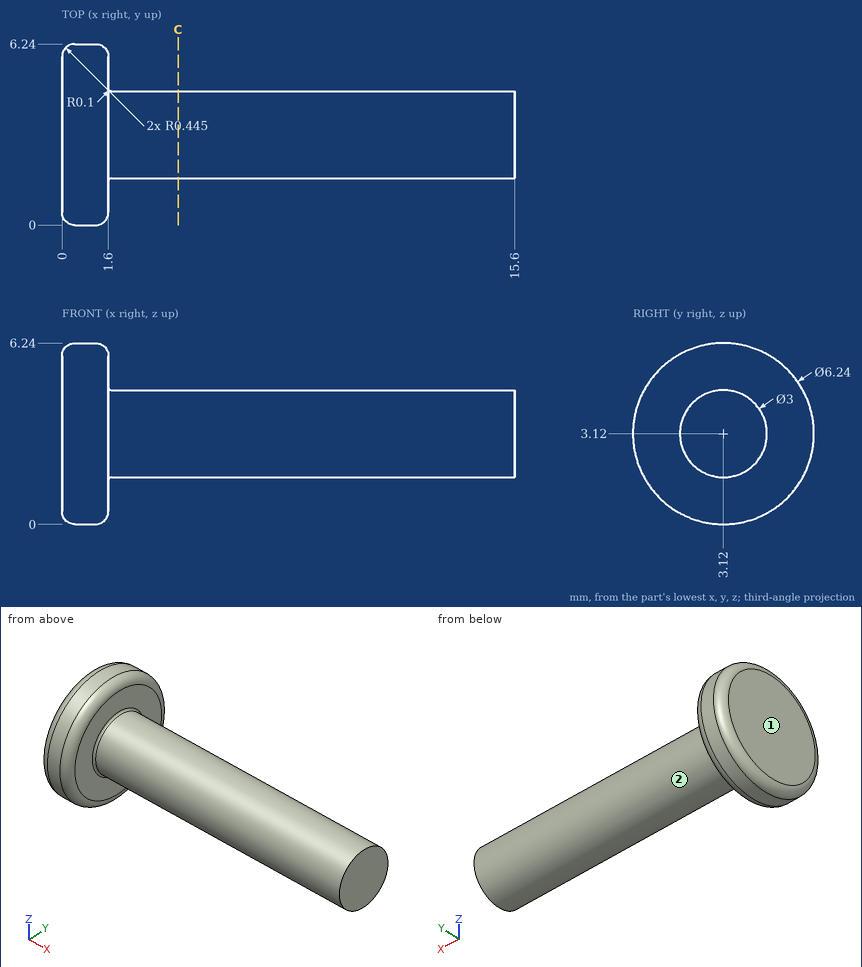
Geometry check sheet. Reference: drawing and pictorial views, mm from the part's lowest x, y, z. A direction names the side the tool comes from. Round coordinates to 2 decimals unless told otherwise and drop trailing zeros. Order: outer loops, then holes, each group sorted by start corner. A loop starts at its lowest first (then second) coordinate and runs counter-clockwise, first axis right, second up. Notation, with made-up numbers: M 10.25,-12 L 24.25,-12 A19 cw 24.25,3 Z; hole C 20,63.25 d5. An arc over 180 degrees is marked long. Write item = value, one per line.
Q1. Section check C-C (x = 4). Enter the section's corners in (y, z).
Answer block:
outline = C 3.12,3.12 d3
Q2. Set-up check for the marked faces 1 and 2: record each of +Z, -Z, +X, -X, +Y, -Y from which the full face is reachable in a straight line by a thin tool's end or side.
Answer block:
face_1 = +Z, -Z, -X, +Y, -Y
face_2 = +X
Q3. Depth check by flat-ended pin: pin 1 Ø2 at (x, y) = (10.5, 3) entering from +Z; pin 2 Ø1 at (x, z) = (8, 3.5) entering from +Y. Enter the tip coordinate at first touch or a pass-through.
Answer block:
pin_1 = 4.62
pin_2 = 4.62
Q4. Scan lines: line 1 (X direction, y = 4.5, z = 2); line 2 (Z direction, x = 9, y = 1.75); line 3 (Z direction, x = 7.25, y = 2.5). Record each from-to range of solid material in increasing order.
Answer block:
line_1 = 0 to 1.6
line_2 = 2.51 to 3.73
line_3 = 1.75 to 4.49
